from build123d import *

# Parameters (mm, degrees)
BASE_EXTRUDE_DEPTH = 10
SKETCH4_W          = 0.8
SKETCH4_H          = 11.856406461
CHAMFER_2_SIZE     = 1.6
FILLET_2_R         = 0.6


with BuildPart() as part:
    # Sketch1 → Base-Extrude (new body)
    with BuildSketch(Plane(origin=(0, 0, 0), x_dir=(0, 0, -1), z_dir=(1, 0, 0))):
        Polygon((12, 6.92820323), (12, -6.92820323), (0, -13.856406461), (-12, -6.92820323), (-12, 6.92820323), (0, 13.856406461), align=None)
    extrude(amount=BASE_EXTRUDE_DEPTH)

    # Sketch2 → Boss-Revolve1 (revolve)
    with BuildSketch(Plane.XY, mode=Mode.PRIVATE) as boss_revolve1_sk:
        Polygon((0, 0), (48, 0), (48, 6.268), (48, 8), (27.8072, 8), (0, 8), align=None)
    revolve(boss_revolve1_sk.sketch.rotate(Axis((0, 0, 0), (1, 0, 0)), 90), axis=Axis((0, 0, 0), (1, 0, 0)))

    # Sketch3 → Cut-Revolve1 (revolve, cut)
    with BuildSketch(Plane.XY):
        Polygon((0, 12), (3.958548116, 18.856406461), (3.958548116, 23.856406461), (-10, 23.856406461), (-10, 12), align=None)
    revolve(axis=Axis((0, 0, 0), (1, 0, 0)), mode=Mode.SUBTRACT)

    # Sketch5 → Cut-Revolve2 (revolve, cut)
    with BuildSketch(Plane.XY):
        Polygon((10, 12), (6.041451884, 18.856406461), (6.041451884, 23.856406461), (16.041451884, 23.856406461), (16.041451884, 12), align=None)
    revolve(axis=Axis((0, 0, 0), (1, 0, 0)), mode=Mode.SUBTRACT)

    # Sketch4 → Cut-Revolve3 (revolve, cut)
    with BuildSketch(Plane.XY, mode=Mode.PRIVATE) as cut_revolve3_sk:
        with Locations((9.6, 17.928203231)):
            Rectangle(SKETCH4_W, SKETCH4_H)
    revolve(cut_revolve3_sk.sketch.rotate(Axis((0, 0, 0), (1, 0, 0)), 270), axis=Axis((0, 0, 0), (1, 0, 0)), mode=Mode.SUBTRACT)

    # Chamfer 2
    chamfer_2_edges = [part.edges().sort_by_distance(p)[0] for p in [
        (48, 0, -8),
    ]]
    chamfer(chamfer_2_edges, length=CHAMFER_2_SIZE)

    # Fillet 2
    fillet_2_edges = [part.edges().sort_by_distance(p)[0] for p in [
        (10, 0, -8),
    ]]
    fillet(fillet_2_edges, radius=FILLET_2_R)


solid = part.part
Read the model definition and answer for the solid it produces. Units are mm, in the model's axes. A direction names the side the tool comes from. Round coordinates to 2 decimals unless told otherwise and drop trailing zeros. Write each loop counter-clockwise with the first axis right and the second up, starting at its lowest first coordinate (ties: lowest second). Pieces come first, ordered by that corner, then holes.
1. Straight lines are drawn through the part: L1, parallel to X at y = -10.5, z = -2; L2, parallel to Z at x = 22, y = 4; L3, parallel to Y at x = 24.5, z = 6.75. For each, find the intervals that lie inside material, in ascending order.
2. Which of the six approach directions +Z, -Z, +X, -X, +Y, -Y give full straight-line access (tool end or side, diameter ignored) to faces 1 (the face through (9.2, 6, 11)), 2 (the face through (9.2, -6, 11)), 3 (the face through (9.2, 6, -11))?
3. The part is cut by section A-A, the plane x = 7. Determine the outline of the cut face in (y, z), then the cut area to 3 significant figures.
4. The part is cut by section B-B, the plane x = 33. Determine the outline of the cut face in (y, z).
5. Given pin 1 Ø5 at (x, z) = (35, 0) entering from +Y; pin 2 Ø3 at (y, z) = (-3.5, -8) entering from +X; pin 3 Ø1 at (x, z) = (7, 5) entering from +Y, each flat-ended and moving along its own axis, determine where each tip first touches the part or whether it passes through.
Values:
1. L1: x = 0 to 10
1. L2: z = -6.93 to 6.93
1. L3: y = -4.29 to 4.29
2. face 1: +Z, +X, +Y
2. face 2: +Z, +X, -Y
2. face 3: -Z, +X, +Y
3. outline: (-13.86, 0) - (-6.93, -12) - (6.93, -12) - (13.86, 0) - (6.93, 12) - (-6.93, 12) - close
3. area: 499 mm2
4. outline: circle Ø16 at (0, 0)
5. pin 1: stops at y = 8
5. pin 2: stops at x = 47.17
5. pin 3: stops at y = 11.26
